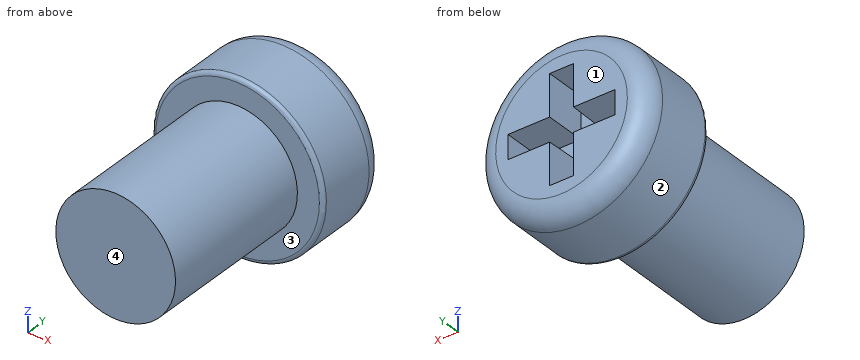
```python
from build123d import *

# Parameters (mm, degrees)
SKETCH1_R           = 2.15
BOSS_EXTRUDE1_DEPTH = 2
SKETCH2_R           = 1.5
BOSS_EXTRUDE2_DEPTH = 4
FILLET1_R           = 0.5
FILLET2_R           = 0.1
CUT_EXTRUDE1_DEPTH  = 1
CUT_EXTRUDE1_DRAFT  = -1


with BuildPart() as part:
    # Sketch1 → Boss-Extrude1 (new body)
    with BuildSketch(Plane(origin=(0, 0, 0), x_dir=(1, 0, 0), z_dir=(0, 1, 0))):
        with Locations(Location((0, 0, 0), (0, 0, 270))):
            Circle(SKETCH1_R)
    extrude(amount=BOSS_EXTRUDE1_DEPTH)

    # Sketch2 → Boss-Extrude2 (add)
    with BuildSketch(Plane.XZ):
        with Locations(Location((0, 0, 0), (0, 0, 90))):
            Circle(SKETCH2_R)
    extrude(amount=BOSS_EXTRUDE2_DEPTH)

    # Fillet1
    fillet1_edges = [part.edges().sort_by_distance(p)[0] for p in [
        (0, 2, -2.15),
    ]]
    fillet(fillet1_edges, radius=FILLET1_R)

    # Fillet2
    fillet2_edges = [part.edges().sort_by_distance(p)[0] for p in [
        (0, 0, -2.15),
    ]]
    fillet(fillet2_edges, radius=FILLET2_R)


with BuildPart() as cut_extrude1_tool:
    # Sketch3 → Cut-Extrude1 (with draft: the straight prism first)
    with BuildSketch(Plane(origin=(0, 2, 0), x_dir=(1, 0, 0), z_dir=(0, 1, 0))):
        Polygon((0.296573117, 0.3), (0.296573117, 1.336133674), (-0.303426883, 1.336133674), (-0.303426883, 0.3), (-1.340662941, 0.3), (-1.340662941, -0.3), (-0.303426883, -0.3), (-0.303426883, -1.336133674), (0.296573117, -1.336133674), (0.296573117, -0.3), (1.340662941, -0.3), (1.340662941, 0.3), align=None)
    extrude(amount=-CUT_EXTRUDE1_DEPTH)
    # Cut-Extrude1: the draft: its side faces are tilted about the plane it starts from
    cut_extrude1_sides = [cut_extrude1_tool.faces().sort_by_distance(p)[0] for p in [
        (0.296573117, 1.5, -0.818066837),
        (-0.003426883, 1.5, -1.336133674),
        (-0.303426883, 1.5, -0.818066837),
        (-0.822044912, 1.5, -0.3),
        (-1.340662941, 1.5, 0),
        (-0.822044912, 1.5, 0.3),
        (-0.303426883, 1.5, 0.818066837),
        (-0.003426883, 1.5, 1.336133674),
        (0.296573117, 1.5, 0.818066837),
        (0.818618029, 1.5, 0.3),
        (1.340662941, 1.5, 0),
        (0.818618029, 1.5, -0.3),
    ]]
    draft(cut_extrude1_sides, Plane(origin=(0, 2, 0), x_dir=(1, 0, 0), z_dir=(0, 1, 0)), CUT_EXTRUDE1_DRAFT)


with BuildPart() as part_1:
    add(part.part)

    # Cut-Extrude1: cut by cut_extrude1_tool
    add(cut_extrude1_tool.part, mode=Mode.SUBTRACT)


solid = part_1.part
```
Geometry: final body of the model. Coordinates: model frame, mm. Face numbers are marked on the shaded views. A direction names the side the tool comes from. Round coordinates to 2 decimals unless told otherwise and drop trailing zeros. Order: outer loops, then holes, each group sorted by start corner. A loop starts at its lowest first (then second) coordinate and runs counter-clockwise, first axis right, second up. Notation, with made-up numbers: (-25, -5.5) -> (7, -5.5) arc R24 ccw to (7, 33.5) -> close; hole circle Ø9 at (67.25, 69.5). An arc over 180 degrees is marked (long way). Use CSV: the item, a comma, the result in double quotes. Start each with the question number.
1) Section C-C (y = 0.2). Return the cut outline in (x, z).
2) Draft query along Z for the marked faces 1 and 2. Return one class per face: +Z half, -Z half, draft (parallel to the pull), parting line (faces both ways), or undercut.
3) Section B-B (x = 0). Return the cut outline in (y, z), and give its area (3 significant figures).
4) Set-up query: the marked faces 3 and 4. Return all of +Z, -Z, +X, -X, +Y, -Y with unobstructed straight access to the full face (end or side cutting, diameter ignored); none if empty.
5) Section D-D (y = -0.6). Return the cut outline in (x, z), and give its area (3 significant figures).
6) Material intervals for line 1 along Y through (x, z) = (-0.8, 0.2); line 2 along X through (y, z) = (1.05, -0.5); line 3 along Z through (x, y) = (-1.1, 1.05), sorted ascending. Write a range as from..to.
7) Section A-A (z = 0). Return the cut outline in (x, y), and give its area (3 significant figures).
Returned:
1,outline,"circle Ø4.3 at (0, 0)"
2,face 1,"draft"
2,face 2,"parting line"
3,outline,"(-4, -1.5) -> (0, -1.5) -> (0, -2.05) arc R0.1 ccw to (0.1, -2.15) -> (1.5, -2.15) arc R0.5 ccw to (2, -1.65) -> (2, -1.34) -> (1, -1.32) -> (1, 1.32) -> (2, 1.34) -> (2, 1.65) arc R0.5 ccw to (1.5, 2.15) -> (0.1, 2.15) arc R0.1 ccw to (0, 2.05) -> (0, 1.5) -> (-4, 1.5) -> close"
3,area,"17.8 mm²"
4,face 3,"-Y"
4,face 4,"+Z, -Z, +X, -X, -Y"
5,outline,"circle Ø3 at (0, 0)"
5,area,"7.07 mm²"
6,line 1,"y = -4..1"
6,line 2,"x = -2.09..-0.29, 0.28..2.09"
6,line 3,"z = -1.85..-0.28, 0.28..1.85"
7,outline,"(-2.15, 0.1) arc R0.1 ccw to (-2.05, 0) -> (-1.5, 0) -> (-1.5, -4) -> (1.5, -4) -> (1.5, 0) -> (2.05, 0) arc R0.1 ccw to (2.15, 0.1) -> (2.15, 1.5) arc R0.5 ccw to (1.65, 2) -> (1.34, 2) -> (1.32, 1) -> (-1.32, 1) -> (-1.34, 2) -> (-1.65, 2) arc R0.5 ccw to (-2.15, 1.5) -> close"
7,area,"17.8 mm²"
